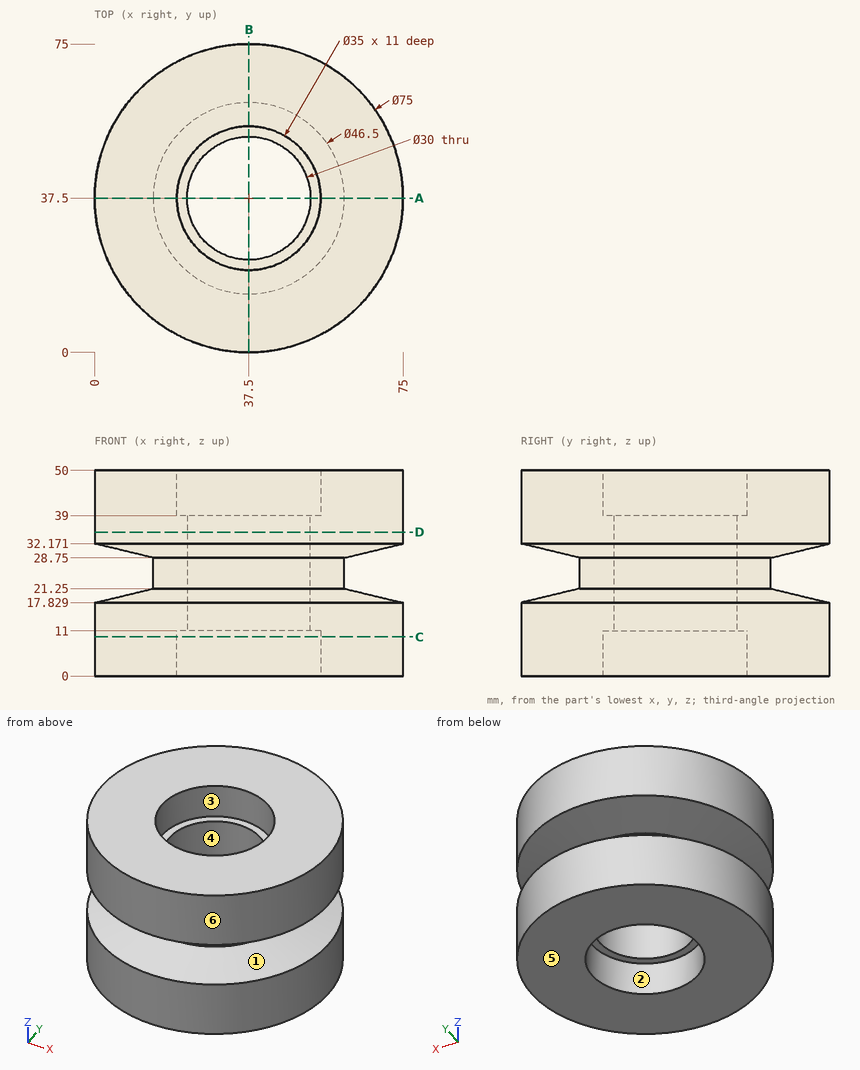
Design review of the part shown in the three views and the two pictorial views. Dimensions are in mm from the part's minimum x, y and z. A direction names the side the tool comes from. Round coordinates to 2 decimals unless told otherwise and drop trailing zeros. Order: outer loops, then holes, each group sorted by start corner. A loop starts at its lowest first (then second) coordinate and runs counter-clockwise, first axis right, second up.
Item 1: To check wall thickness, follow probe 1 along Y at (x, z) = (37.5, 43.5); probe 2 along X at (y, z) = (37.5, 17.25). State the ranges of each line that lie inside material, in increasing order.
Working result:
probe 1: y = 0 to 20, 55 to 75
probe 2: x = 0 to 22.5, 52.5 to 75
Item 2: Add section C-C, the plane z = 9.5. State the section outline as (x, y) points, and give its area (3 significant figures).
Working result:
outline: circle Ø75 at (37.5, 37.5); hole circle Ø35 at (37.5, 37.5)
area: 3,460 mm2
Item 3: Add section D-D, the plane z = 35. State the section outline as (x, y) points.
Working result:
outline: circle Ø75 at (37.5, 37.5); hole circle Ø30 at (37.5, 37.5)
Item 4: Machinability: for the marked faces 1, 2 and 3, which of the approach directions +Z, -Z, +X, -X, +Y, -Y give a long, thin tool a straight path to every point of the face, cutting with its end or side? Answer none if there is none.
Working result:
face 1: none
face 2: -Z
face 3: +Z
Item 5: For pin 1 (12 mm diameter, centred on y = 64, z = 13.5, fed in from +X); pin 2 (8 mm diameter, centred on x = 35, z = 32.5, fed in from +Y); pin 3 (6 mm diameter, centred on x = 61, z = 38.5, fed in from -Y), all flat-tipped, find the tip position at first contact; note any pin that passes through.
Working result:
pin 1: stops at x = 68.9
pin 2: stops at y = 75
pin 3: stops at y = 6.1
Item 6: Add section A-A, the plane y = 37.5. State the section outline as (x, z) points.
Working result:
outline: (0, 0) - (20, 0) - (20, 11) - (22.5, 11) - (22.5, 39) - (20, 39) - (20, 50) - (0, 50) - (0, 32.17) - (14.25, 28.75) - (14.25, 21.25) - (0, 17.83) - close; (52.5, 11) - (55, 11) - (55, 0) - (75, 0) - (75, 17.83) - (60.75, 21.25) - (60.75, 28.75) - (75, 32.17) - (75, 50) - (55, 50) - (55, 39) - (52.5, 39) - close
Item 7: Draft analysis for pull direction X (two halves, no side actions). For the marked faces 4, 5 and 6, state which applies: released by +X, released by -X, zero draft, split by the parting line, or undercut.
Working result:
face 4: undercut
face 5: zero draft
face 6: split by the parting line
